Work out the finished part from the listing and answer in its coordinate system (mm). A direction names the side the tool comes from. Coordinates: 2 decimals unless noted, no trailing zeros. Order: outer loops, then holes, each group sorted by start corner. A loop starts at its lowest first (then second) coordinate and runs counter-clockwise, first axis right, second up. Notation, with made-up numbers: M -20,-19 L 4,-19 A29 ccw 4,12 Z; hole C 67.5,79 d10. An arc over 180 degrees is marked long. Use a Markdown table: item, result.
from build123d import *

# Parameters (mm, degrees)
BOSS_EXTRUDE1_DEPTH   = 30
FILLET1_R             = 3
M8X1_0_TAPPED_HOLE1_D = 7
CUT_EXTRUDE1_DEPTH    = 39.619021662
CUT_EXTRUDE2_DEPTH    = 3.3


with BuildPart() as part:
    # Sketch1 → Boss-Extrude1 (new body)
    with BuildSketch(Plane(origin=(0, 0, 0), x_dir=(1, 0, 0), z_dir=(0, 1, 0))):
        with BuildLine():
            Line((-22.5, 76.770762664), (-22.5, 86))
            Line((-22.5, 86), (22.5, 86))
            Line((22.5, 86), (22.5, 76.770762664))
            ThreePointArc((22.5, 76.770762664), (0, 80), (-22.5, 76.770762664))
        make_face()
    extrude(amount=BOSS_EXTRUDE1_DEPTH)

    # Fillet1
    fillet1_edges = [part.edges().sort_by_distance(p)[0] for p in [
        (22.5, 30, -81.385381332),
        (22.5, 0, -81.385381332),
        (-22.5, 0, -81.385381332),
        (-22.5, 30, -81.385381332),
    ]]
    fillet(fillet1_edges, radius=FILLET1_R)

    # M8x1.0 Tapped Hole1 (through all)
    with Locations(Plane(origin=(0, 0, -86), x_dir=(-1, 0, 0), z_dir=(0, 0, -1))):
        with Locations((0, 15)):
            Hole(M8X1_0_TAPPED_HOLE1_D / 2)

    # Sketch4 → Cut-Extrude1 (cut, through all)
    with BuildSketch(Plane(origin=(0, 0, -86), x_dir=(-1, 0, 0), z_dir=(0, 0, -1))):
        with BuildLine():
            Line((-12.75, 20), (-12.75, 10))
            ThreePointArc((-12.75, 10), (-14.5, 8.25), (-16.25, 10))
            Line((-16.25, 10), (-16.25, 20))
            ThreePointArc((-16.25, 20), (-14.5, 21.75), (-12.75, 20))
        make_face()
        with BuildLine():
            Line((16.25, 20), (16.25, 10))
            ThreePointArc((16.25, 10), (14.5, 8.25), (12.75, 10))
            Line((12.75, 10), (12.75, 20))
            ThreePointArc((12.75, 20), (14.5, 21.75), (16.25, 20))
        make_face()
    extrude(amount=-CUT_EXTRUDE1_DEPTH, mode=Mode.SUBTRACT)

    # Sketch5 → Cut-Extrude2 (cut)
    with BuildSketch(Plane(origin=(0, 0, -86), x_dir=(-1, 0, 0), z_dir=(0, 0, -1))):
        with BuildLine():
            Line((-11.5, 20), (-11.5, 10))
            ThreePointArc((-11.5, 10), (-14.5, 7), (-17.5, 10))
            Line((-17.5, 10), (-17.5, 20))
            ThreePointArc((-17.5, 20), (-14.5, 23), (-11.5, 20))
        make_face()
        with BuildLine():
            Line((17.5, 20), (17.5, 10))
            ThreePointArc((17.5, 10), (14.5, 7), (11.5, 10))
            Line((11.5, 10), (11.5, 20))
            ThreePointArc((11.5, 20), (14.5, 23), (17.5, 20))
        make_face()
    extrude(amount=-CUT_EXTRUDE2_DEPTH, mode=Mode.SUBTRACT)


solid = part.part
(1) Straight lines are drawn through the part: L1, parallel to X at y = 15, z = -81.5; L2, parallel to X at y = 15, z = -83.75; L3, parallel to Y at x = -14.5, z = -79.5. For each, find the intervals that lie inside material, in ascending order.
Conclusion:
| item | result |
|---|---|
| L1 | -22.5 to -16.25, -12.75 to -3.5, 3.5 to 12.75, 16.25 to 22.5 |
| L2 | -22.5 to -17.5, -11.5 to -3.5, 3.5 to 11.5, 17.5 to 22.5 |
| L3 | 0 to 8.25, 21.75 to 30 |
(2) Which of the six approach directions +Z, -Z, +X, -X, +Y, -Y give full straight-line access (tool end or side, diameter ignored) to faces 1 (the cylindrical face through (21.64, 29.1, -81.32)), 2 (the flat face through (-17.5, 15, -84)), 3 (the flat face through (-16.25, 15, -81))?
Conclusion:
| item | result |
|---|---|
| face 1 | +Z, -Z, +X, +Y |
| face 2 | -Z |
| face 3 | +Z, -Z |
(3) Given P1, Ø6.5, axis at x = -14, y = 11.5, coming from the -Z side; P2, Ø3, axis at x = 13.5, y = 15.5, coming from the -Z side, each flat-ended and moving along its own axis, determine where each tip first touches the part or whether it passes through.
Conclusion:
| item | result |
|---|---|
| P1 | z = -86 |
| P2 | z = -82.7 |
(4) A cutting plane is placed at B-B (y = 15). Determine the outline of the cut face in (x, z), then the cut area to 3 significant figures.
Conclusion:
| item | result |
|---|---|
| outline | M -22.5,-86 L -17.5,-86 L -17.5,-82.7 L -16.25,-82.7 L -16.25,-78.33 A80 cw -22.5,-76.77 Z; M -12.75,-82.7 L -11.5,-82.7 L -11.5,-86 L -3.5,-86 L -3.5,-79.92 A80 cw -12.75,-78.98 Z; M 3.5,-86 L 11.5,-86 L 11.5,-82.7 L 12.75,-82.7 L 12.75,-78.98 A80 cw 3.5,-79.92 Z; M 16.25,-82.7 L 17.5,-82.7 L 17.5,-86 L 22.5,-86 L 22.5,-76.77 A80 cw 16.25,-78.33 Z |
| area | 208 mm2 |
(5) Determine the mould class of faces 4 (the flat face through (0, 11, -86)), 5 (the flat face through (0, 30, -83)), 6 (the flat face through (17.5, 15, -84)) for opening direction Y: pulls with the +Y half, pulls with the -Y half, needs draft (parallel to the pull), parting line crosses it, or undercut.
Conclusion:
| item | result |
|---|---|
| face 4 | needs draft |
| face 5 | pulls with the +Y half |
| face 6 | undercut |
(6) A cutting plane is placed at C-C (z = -82). Determine the outline of the cut face in (x, y).
Conclusion:
| item | result |
|---|---|
| outline | M -22.5,3 A3 ccw -19.5,0 L 19.5,0 A3 ccw 22.5,3 L 22.5,27 A3 ccw 19.5,30 L -19.5,30 A3 ccw -22.5,27 Z; hole M -16.25,10 A1.75 ccw -12.75,10 L -12.75,20 A1.75 ccw -16.25,20 Z; hole C 0,15 d7; hole M 12.75,10 A1.75 ccw 16.25,10 L 16.25,20 A1.75 ccw 12.75,20 Z |
(7) A cutting plane is placed at D-D (x = -14.5). Determine the outline of the cut face in (y, z).
Conclusion:
| item | result |
|---|---|
| outline | M 0,-86 L 7,-86 L 7,-82.7 L 8.25,-82.7 L 8.25,-78.67 L 0,-78.67 Z; M 21.75,-82.7 L 23,-82.7 L 23,-86 L 30,-86 L 30,-78.67 L 21.75,-78.67 Z |
(8) A cutting plane is placed at A-A (x = 0). Determine the outline of the cut face in (y, z).
Conclusion:
| item | result |
|---|---|
| outline | M 0,-86 L 11.5,-86 L 11.5,-80 L 0,-80 Z; M 18.5,-86 L 30,-86 L 30,-80 L 18.5,-80 Z |
